from build123d import *

# Parameters (mm, degrees)
HOLE_WIZARD_M3_1_REACH  = 21.894
HOLE_WIZARD_M3_1_BORE_R = 1.25


with BuildPart() as part:
    # 草图1 → 旋转1 (revolve)
    with BuildSketch(Plane.XY, mode=Mode.PRIVATE) as revolve_1_sk:
        Polygon((9.5, 9.117025796), (2.5, 9.117025796), (2.5, 1.117025796), (9.5, 1.117025796), (9.5, 2.117025796), (7.5, 2.117025796), (7.5, 8.117025796), (9.5, 8.117025796), align=None)
    revolve(revolve_1_sk.sketch.rotate(Axis((0, 18.913531016, 0), (0, -1, 0)), 90), axis=Axis((0, 18.913531016, 0), (0, -1, 0)))

    # M3 螺纹孔1 bore (on position points) → M3 螺纹孔1 (cut, up to next)
    with BuildSketch(Plane(origin=(0.019511296, 5.135461688, 7.499974621), x_dir=(0.999996616077, 0, -0.002601506145), z_dir=(0.002601506145, 0, 0.999996616077)), mode=Mode.PRIVATE) as hole_wizard_m3_1_sk1:
        Circle(HOLE_WIZARD_M3_1_BORE_R)
    hole_wizard_m3_1_tool1 = extrude(hole_wizard_m3_1_sk1.sketch, amount=-HOLE_WIZARD_M3_1_REACH, mode=Mode.PRIVATE) & part.part
    add(hole_wizard_m3_1_tool1.solids().sort_by_distance((0.019511, 5.135462, 7.499975))[0], mode=Mode.SUBTRACT)


solid = part.part
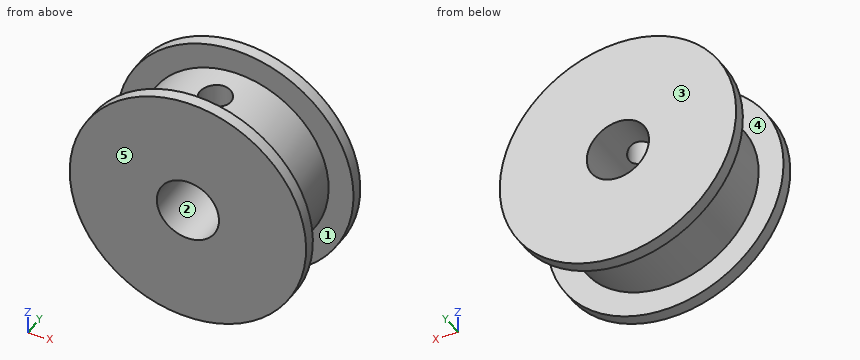
Could you check a few things on this model? Use its own coordinates, in mm. Face numbers are marked on the shaded views. A direction names the side the tool comes from. Coordinates: 2 decimals unless noted, no trailing zeros. Write each loop counter-clockwise with the first axis right and the second up, starting at its lowest first coordinate (ties: lowest second). Pieces come first, ordered by that corner, then holes. Notation, with made-up numbers: (-4, -7) - (50, -7) arc R21 cw to (50, 12) - close; hole circle Ø3 at (57.25, 63). An arc over 180 degrees is marked (long way). Put each result on its own line as item: value. Start each with the question number.
Q1. I want a section at D-D on x = 4.25. Write out the boundary of the cut face in (y, z), plus the area to 3 significant figures.
Q2. I want a section at B-B on y = 7.25. Write out the boundary of the cut face in (x, z).
Q3. I'm going to push flat-ended pins straight in: P1, Ø4.5, axis at x = 0, z = 0, coming from the +Y side; P2, Ø1.5, axis at y = 3, z = -5.5, coming from the +X side; P3, Ø2, axis at x = 7, y = 4.5, coming from the +Z side. Where does each tip first touch, or does it pass through?
Q4. Please list where these lines run through material, in increasing order: L1, parallel to Y at x = -1.5, z = -8.5; L2, parallel to Z at x = 0, y = 2.25.
Q5. Which directions (+Z, -Z, +X, -X, +Y, -Y) give clear straight access to the entire face, cutting with the end or side of a thin tool? Please do the marked faces 1 and 2.
Q6. I want a section at C-C on x = -8. Write out the boundary of the cut face in (y, z).
Q7. Thinking about a two-plate mould opening in Y: for the marked faces 3, 4 and 5, which applies, pulls with the +Y half, pulls with the -Y half, needs draft (parallel to the pull), parting line crosses it, or undercut?
Q8. I want a section at A-A on z = 0. Write out the boundary of the cut face in (x, y), plus the area to 3 significant figures.
Checks:
1. outline: (1.12, -8.5) - (2.12, -8.5) - (2.12, -6.18) - (8.12, -6.18) - (8.12, -8.5) - (9.12, -8.5) - (9.12, 8.5) - (8.12, 8.5) - (8.12, 6.18) - (2.12, 6.18) - (2.12, 8.5) - (1.12, 8.5) - close
1. area: 108 mm²
2. outline: circle Ø15 at (0, 0); hole circle Ø5 at (0, 0)
3. P1: through
3. P2: x = 5.8
3. P3: z = 4.5
4. L1: 1.12 to 2.12, 8.12 to 9.12
4. L2: -7.5 to -2.5, 2.5 to 7.5
5. face 1: none
5. face 2: +Y, -Y
6. outline: (1.12, -5.12) - (2.12, -5.12) - (2.12, 5.12) - (1.12, 5.12) - close; (8.12, -5.12) - (9.12, -5.12) - (9.12, 5.12) - (8.12, 5.12) - close
7. face 3: pulls with the +Y half
7. face 4: undercut
7. face 5: pulls with the -Y half
8. outline: (-9.5, 1.12) - (-2.5, 1.12) - (-2.5, 9.12) - (-9.5, 9.12) - (-9.5, 8.12) - (-7.5, 8.12) - (-7.5, 2.12) - (-9.5, 2.12) - close; (2.5, 1.12) - (9.5, 1.12) - (9.5, 2.12) - (7.5, 2.12) - (7.5, 8.12) - (9.5, 8.12) - (9.5, 9.12) - (2.5, 9.12) - close
8. area: 88.0 mm²
